```python
from build123d import *

# Parameters (mm, degrees)
BOSS_EXTRUDE1_START = -2.8
SKETCH4_R           = 0.75
BOSS_EXTRUDE1_DEPTH = 2.8
SKETCH5_R           = 4.582903769
SKETCH5_R_2         = 3.5
CUT_EXTRUDE1_DEPTH  = 1
CUT_EXTRUDE1_DRAFT  = -55
CHAMFER1_SIZE       = 0.4


with BuildPart() as part:
    # Sketch3 → Revolve1 (revolve)
    with BuildSketch(Plane(origin=(0, 0, 0), x_dir=(0, 0, -1), z_dir=(1, 0, 0)), mode=Mode.PRIVATE) as revolve1_sk:
        Polygon((0, 2), (-2.8, 2), (-2.8, 0.75), (20, 0.75), (20, 2), align=None)
    revolve(revolve1_sk.sketch.rotate(Axis((0, 0, 2.8), (0, 0, -1)), 180), axis=Axis((0, 0, 2.8), (0, 0, -1)))

    # Sketch4 → Boss-Extrude1 (add)
    with BuildSketch(Plane.XY.offset(2.8).offset(BOSS_EXTRUDE1_START)):
        Polygon((2.020725942, 3.5), (-2.020725942, 3.5), (-4.041451884, 0), (-2.020725942, -3.5), (2.020725942, -3.5), (4.041451884, 0), align=None)
        with Locations(Location((0, 0, 0), (0, 0, 270))):
            Circle(SKETCH4_R, mode=Mode.SUBTRACT)
    extrude(amount=BOSS_EXTRUDE1_DEPTH)


with BuildPart() as cut_extrude1_tool:
    # Sketch5 → Cut-Extrude1 (with draft: the straight prism first)
    with BuildSketch(Plane.XY.offset(2.8)):
        Circle(SKETCH5_R)
        Circle(SKETCH5_R_2, mode=Mode.SUBTRACT)
    extrude(amount=-CUT_EXTRUDE1_DEPTH)
    # Cut-Extrude1: the draft: its side faces are tilted about the plane it starts from
    cut_extrude1_sides = [cut_extrude1_tool.faces().sort_by_distance(p)[0] for p in [
        (-4.582903769, 0, 2.3),
        (-3.5, 0, 2.3),
    ]]
    draft(cut_extrude1_sides, Plane.XY.offset(2.8), CUT_EXTRUDE1_DRAFT)


with BuildPart() as part_1:
    add(part.part)

    # Cut-Extrude1: cut by cut_extrude1_tool
    add(cut_extrude1_tool.part, mode=Mode.SUBTRACT)

    # Chamfer1
    chamfer1_edges = [part_1.edges().sort_by_distance(p)[0] for p in [
        (0, 2, -20),
    ]]
    chamfer(chamfer1_edges, length=CHAMFER1_SIZE)


solid = part_1.part
```
The listing builds one solid part. Answer for the finished solid, in the listing's coordinates (mm). A direction names the side the tool comes from. Round coordinates to 2 decimals unless told otherwise and drop trailing zeros. Loops run counter-clockwise (first coordinate to the right, second up) from the corner with the lowest first, then second, coordinate; pieces in that order, holes last. Notation, with made-up numbers: (-20, 58) -> (-7, 58) arc R27 ccw to (-7, 87) -> close; hole circle Ø7 at (-35.5, 54). An arc over 180 degrees is marked (long way). Use one line per item in the form item = value.
1. Find the intervals of material crossed by probe 1 along X at (y, z) = (0, -11.5); probe 2 along Z at (x, y) = (1.25, 2.75); probe 3 along Y at (x, z) = (-0.5, -0.25), in increasing order. Write a range as [from, to].
Answer key:
probe_1 = [-2, -0.75], [0.75, 2]
probe_2 = [0, 2.8]
probe_3 = [-1.94, -0.56], [0.56, 1.94]
2. The part is cut by section A-A on z = 0.5. Determine the outline of the cut face in (x, y).
Answer key:
outline = (-4.04, 0) -> (-2.02, -3.5) -> (2.02, -3.5) -> (4.04, 0) -> (2.02, 3.5) -> (-2.02, 3.5) -> close; hole circle Ø1.5 at (0, 0)
3. For a pull along X with two mould halves and no side action, classify faces 1 (the flat face through (3.045, 1.726, 1.38)), 2 (the cylindrical face through (-0.225, -0.715, -8.76)), 3 (the flat face through (-3.045, -1.725, 1.38)) as released by +X, released by -X, zero draft, split by the parting line, or undercut.
Answer key:
face_1 = released by +X
face_2 = undercut
face_3 = released by -X
4. Flat-ended cylindrical pins translate along their axes: pin 1 Ø1.5 at (x, z) = (-0.5, -5.5) entering from +Y; pin 2 Ø1 at (y, z) = (0, -14.5) entering from +X; pin 3 Ø1 at (x, z) = (1.5, -9) entering from -Y. Find the tip coordinate at first contact, or state that the pin passes through.
Answer key:
pin_1 = 2
pin_2 = 2
pin_3 = -1.73
5. A tool of negligible diameter and unlimited length cuts with its end or side. For faces 4 (the flat face through (2, 2, 0)), 5 (the conical face through (-1.807, 3.147, 2.71)), from which of +Z, -Z, +X, -X, +Y, -Y can it reach the whole face along a straight path? Write none if from no direction.
Answer key:
face_4 = -Z
face_5 = +Z, -X, +Y
